For this review, take the finished solid that the model builds, in its own axes (mm). Give positions to 0.01 mm unless a question says otherwise; leave off trailing zeros. Write each loop counter-clockwise with the first axis right and the second up, starting at its lowest first coordinate (ties: lowest second). Pieces come first, ordered by that corner, then holes. Notation, with made-up numbers: M 78,5.5 L 122,5.5 A20 cw 122,19.5 Z; hole C 32,45 d8. An arc over 180 degrees is marked long. One line per item, written item: value. Start each with the question number.
Item 1: Clearance check with flat-ended pins moving along their axes: pin 1 Ø1.5 at (x, z) = (11.5, 1462) entering from -Y; pin 2 Ø4 at (x, z) = (3.5, 1077.5) entering from -Y (3 decimals); pin 3 Ø10 at (x, y) = (5.5, 26.5) entering from -Z. State where each tip first meets the part, or that it passes through.
Item 2: To check wall thickness, follow probe 1 along Y at (x, z) = (4.75, 900.5) (3 decimals); probe 2 along Z at (x, y) = (8.75, 40); probe 3 along Y at (x, z) = (8.25, 160.5) (3 decimals). State the ranges of each line that lie inside material, in increasing order.
Item 3: Consider section B-B, the plane x = -6.75. Write out the cut boundary in (y, z) (3 decimals), and give its area (3 significant figures).
Item 4: Consider section D-D, the plane z = 1632.5. Write out the cut boundary in (x, y) (3 decimals), and give its area (3 significant figures).
Item 5: Consider section A-A, the plane z = 1022. Write out the cut boundary in (x, y) (3 decimals).
Item 6: Consider section C-C, the plane y = -34.5. Write out the cut boundary in (x, z).
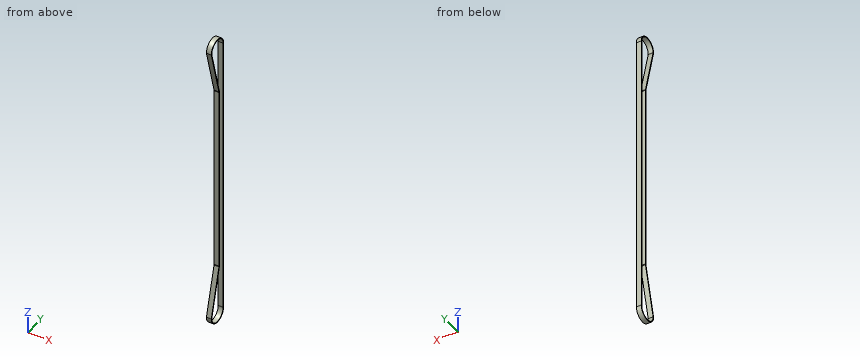
```python
from build123d import *

# Parameters (mm, degrees)
EXTRUDE_1_DEPTH = 15


with BuildPart() as part:
    # 草图2 → 拉伸-薄壁1 (new, symmetric)
    with BuildSketch(Plane(origin=(0, 0, 0), x_dir=(0, 0, -1), z_dir=(1, 0, 0))):
        with BuildLine():
            Line((-295.400568077, 14.914130168), (-0.448465098, -60.793345886))
            ThreePointArc((-0.448465098, -60.793345886), (60.79458647, -0.224234074), (0, 60.795))
            Line((0, 60.795), (-1750, 60.795))
            ThreePointArc((-1750, 60.795), (-1810.79458647, -0.224234074), (-1749.551534902, -60.793345886))
            Line((-1749.551534902, -60.793345886), (-1454.599431923, 14.914130168))
            ThreePointArc((-1454.599431923, 14.914130168), (-1452.317983163, 15.349208075), (-1450, 15.495))
            Line((-1450, 15.495), (-300, 15.495))
            ThreePointArc((-300, 15.495), (-297.682016837, 15.349208075), (-295.400568077, 14.914130168))
        make_face()
        with BuildLine():
            Line((-294.281787339, 19.272837507), (0.125744515, -56.294859564))
            ThreePointArc((0.125744515, -56.294859564), (56.294964891, 0.062872297), (0, 56.295))
            Line((0, 56.295), (-1750, 56.295))
            ThreePointArc((-1750, 56.295), (-1806.294964891, 0.062872297), (-1750.125744515, -56.294859564))
            Line((-1750.125744515, -56.294859564), (-1455.718212661, 19.272837507))
            ThreePointArc((-1455.718212661, 19.272837507), (-1452.881816905, 19.813745174), (-1450, 19.995))
            Line((-1450, 19.995), (-300, 19.995))
            ThreePointArc((-300, 19.995), (-297.118183095, 19.813745174), (-294.281787339, 19.272837507))
        make_face(mode=Mode.SUBTRACT)
    extrude(amount=EXTRUDE_1_DEPTH, both=True)


solid = part.part
```
Model answer:
1. pin 1: stops at y = 12.82
1. pin 2: stops at y = 15.495
1. pin 3: stops at z = -56.87
2. probe 1: y = 15.495 to 19.995, 56.295 to 60.795
2. probe 2: z = -45.78 to -39.61, 1789.61 to 1795.78
2. probe 3: y = -19.712 to -15.066, 56.295 to 60.795
3. outline: M -60.793,0.448 A60.795 ccw long 60.795,0 L 60.795,1750 A60.795 ccw long -60.793,1749.552 L 14.914,1454.599 A18.5 cw 15.495,1450 L 15.495,300 A18.5 cw 14.914,295.401 Z; hole M -56.295,-0.126 A56.295 ccw 56.295,0 L 56.295,1750 A56.295 ccw -56.295,1750.126 L 19.273,1455.718 A23 cw 19.995,1450 L 19.995,300 A23 cw 19.273,294.282 Z
3. area: 17,500 mm2
4. outline: M -15,-30.749 L 15,-30.749 L 15,-26.103 L -15,-26.103 Z; M -15,56.295 L 15,56.295 L 15,60.795 L -15,60.795 Z
4. area: 274 mm2
5. outline: M -15,15.495 L 15,15.495 L 15,19.995 L -15,19.995 Z; M -15,56.295 L 15,56.295 L 15,60.795 L -15,60.795 Z
6. outline: M -15,-50.06 L 15,-50.06 L 15,-44.48 L -15,-44.48 Z; M -15,84.79 L 15,84.79 L 15,102.89 L -15,102.89 Z; M -15,1647.11 L 15,1647.11 L 15,1665.21 L -15,1665.21 Z; M -15,1794.48 L 15,1794.48 L 15,1800.06 L -15,1800.06 Z
